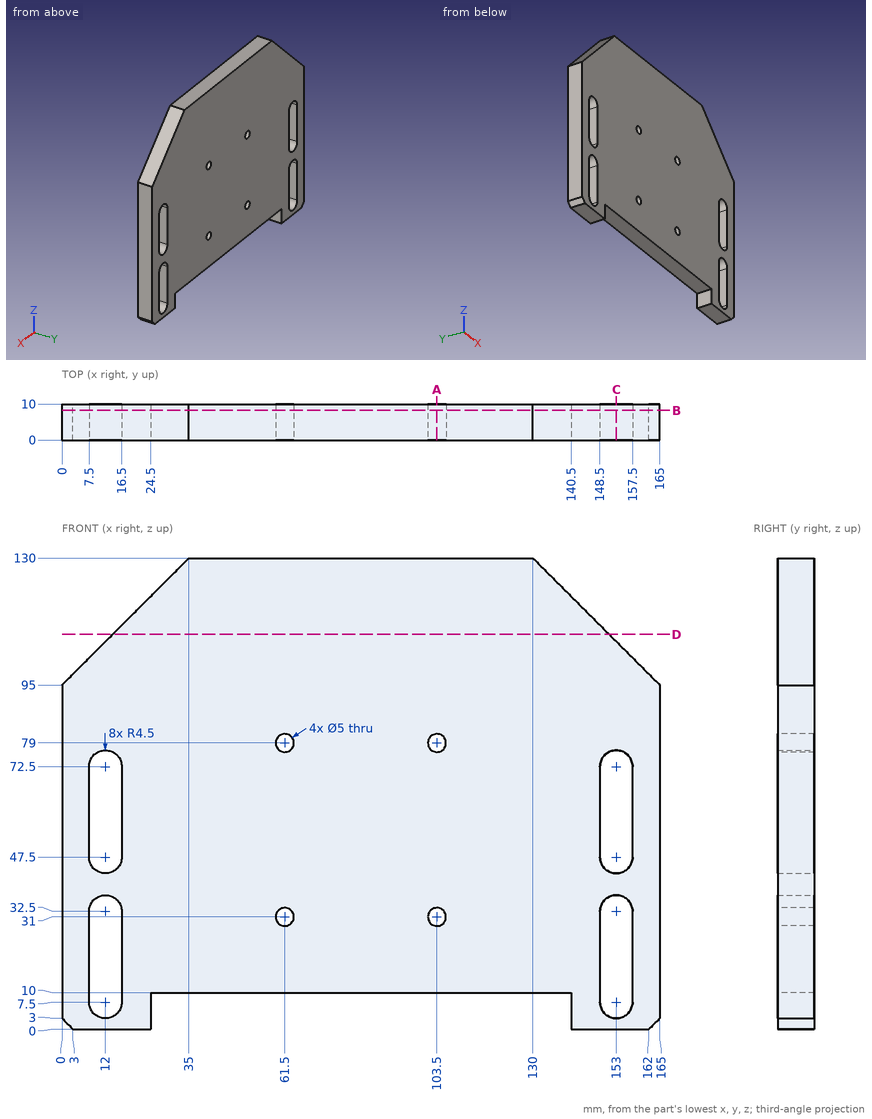
Could you check a few things on this drawing? It's one solid part, dimensions in mm from its lowest x, y, z. Give positions to 0.01 mm unless a question says otherwise; leave off trailing zeros. Order: outer loops, then holes, each group sorted by start corner. A loop starts at its lowest first (then second) coordinate and runs counter-clockwise, first axis right, second up.
1. For pin 1 (6.5 mm diameter, centred on x = 61.5, z = 79, fed in from -Y); pin 2 (3 mm diameter, centred on y = 5, z = 102, fed in from -X); pin 3 (4 mm diameter, centred on x = 138, y = 6, fed in from -Z), each with a flat end and sliding along its axis, tell me the tip position at first contact or that it passes through.
Answers below:
pin 1: stops at y = 0
pin 2: stops at x = 5.5
pin 3: stops at z = 10
2. Suppose I cut it at C-C (x = 153). Write out the boundary of the cut face in (y, z), plus the area to 3 significant figures.
Answers below:
outline: (0, 0) - (10, 0) - (10, 3) - (0, 3) - close; (0, 37) - (10, 37) - (10, 43) - (0, 43) - close; (0, 77) - (10, 77) - (10, 107) - (0, 107) - close
area: 390 mm2
3. Suppose I cut it at B-B (y = 8.25). State how many separate pieces and enclosed holes the cut face has, plus the area to 3 significant figures.
Answers below:
separate pieces: 1
enclosed holes: 8
area: 17,800 mm2
4. I need wall thicknesses on L1, parallel to X at y = 2.25, z = 55; L2, parallel to Z at x = 103.5, y = 4.5; L3, parallel to X at y = 5.5, z = 79. Which ranges of each line are inside material? Lowest first, please.
Answers below:
L1: x = 0 to 7.5, 16.5 to 148.5, 157.5 to 165
L2: z = 10 to 28.5, 33.5 to 76.5, 81.5 to 130
L3: x = 0 to 59, 64 to 101, 106 to 165
5. Suppose I cut it at A-A (x = 103.5). Write out the boundary of the cut face in (y, z), plus the area to 3 significant figures.
Answers below:
outline: (0, 10) - (10, 10) - (10, 28.5) - (0, 28.5) - close; (0, 33.5) - (10, 33.5) - (10, 76.5) - (0, 76.5) - close; (0, 81.5) - (10, 81.5) - (10, 130) - (0, 130) - close
area: 1,100 mm2
6. Suppose I cut it at D-D (z = 109). Write out the boundary of the cut face in (x, y).
Answers below:
outline: (14, 0) - (151, 0) - (151, 10) - (14, 10) - close
